Geometry check sheet. Reference: the model listing, model coordinates, mm. A direction names the side the tool comes from. Coordinates: 2 decimals unless noted, no trailing zeros. Write each loop counter-clockwise with the first axis right and the second up, starting at its lowest first coordinate (ties: lowest second). Pieces come first, ordered by that corner, then holes. Notation, with made-up numbers: M -23.75,-3.75 L 0.25,-3.75 A26 cw 0.25,35.25 Z; hole C 5.5,84.5 d4. An arc over 180 degrees is marked long. Put each result on its own line as item: value. Start each with the question number.
1) Scan lines: line 1 along X through (y, z) = (12, 3.25); line 2 along X through (y, z) = (0.25, -5.5); line 3 along Z through (x, y) = (-3, 11.5). Record each from-to range of solid material in increasing order.
2) Gauge pin test, flat ends, axial feed: pin 1 (3 mm diameter, centred on x = 13, z = -3, fed in from +Y); pin 2 (3 mm diameter, centred on x = -18, y = 0, fed in from -Z); pin 3 (6.5 mm diameter, centred on y = 10, z = 0.5, fed in from +X); pin 4 (2.5 mm diameter, centred on y = 10.5, z = 0, fed in from +X). Record the tip position at first contact, or that the pin passes through.
3) Cross-section at C-C on z = -3.5. Record the cut outline in (x, y), plus the area to 3 significant figures.
4) Mould release check, pull along Z, two halves, no side actions. Record for faces 1 (the flat face through (6, 5, 6.5)), 2 (the flat face through (1.9, 12, 2)), 3 (the flat face through (-5, 5, -6.5)): released by +Z, released by -Z, zero draft, split by the parting line, or undercut.
5) Cross-section at D-D on y = 11.5. Record the cut outline in (x, z), plus the area to 3 significant figures.
6) Cross-section at B-B on x = 16.5. Record the cut outline in (y, z), plus the area to 3 significant figures.
7) Cross-section at A-A on y = 0. Record the cut outline in (x, z).
8) Set-up check for faces 4 (the cylindrical face through (1.21, 8.27, 0.29)), 5 (the flat face through (6.5, 15, 0)), 6 (the flat face through (-6.5, 14, 0)), 7 (the flat face through (-0.5, 9.7, 0.1)), 8 (the cylindrical face through (0.45, -12.49, 2.98)): record each of +Z, -Z, +X, -X, +Y, -Y from which the full face is reachable in a straight line by a thin tool's end or side.
from build123d import *
from build123d.topology import SkipClean

# Parameters (mm, degrees)
EXTRUDE_1_DEPTH     = 6.5
EXTRUDE_START       = -7
SKETCH_2_R          = 2.5
EXTRUDE_2_DEPTH     = 7
SKETCH_3_W          = 1.65
SKETCH_3_H          = 23
CUT_EXTRUDE_START   = 10
CUT_EXTRUDE_1_DEPTH = 10


with BuildPart() as part:
    # 草图1 → 凸台-拉伸1 (new, symmetric)
    with BuildSketch(Plane.XY):
        with BuildLine():
            Line((0.5, 5.979130372), (0.5, 15.5))
            Line((0.5, 15.5), (6.5, 15.5))
            Line((6.5, 15.5), (6.5, 10.677078252))
            ThreePointArc((6.5, 10.677078252), (0, -12.5), (-6.5, 10.677078252))
            Line((-6.5, 10.677078252), (-6.5, 15.5))
            Line((-6.5, 15.5), (-0.5, 15.5))
            Line((-0.5, 15.5), (-0.5, 5.979130372))
            ThreePointArc((-0.5, 5.979130372), (0, -6), (0.5, 5.979130372))
        make_face()
    extrude(amount=EXTRUDE_1_DEPTH, both=True)

    # 草图2 → 凸台-拉伸2 (add)
    # profile 1 of 2: a face of its own
    with BuildSketch(Plane(origin=(0, 0, -6.5), x_dir=(-1, 0, 0), z_dir=(0, 0, -1)).offset(EXTRUDE_START)):
        with BuildLine():
            Line((-23.5, -3), (-5.197687408, -11.368115306))
            ThreePointArc((-5.197687408, -11.368115306), (-12.478245567, -0.737148272), (-6.5, 10.677078252))
            Line((-6.5, 10.677078252), (-23.5, 3))
            Line((-23.5, 3), (-23.5, -3))
        make_face()
        with Locations((-18, 0)):
            Circle(SKETCH_2_R, mode=Mode.SUBTRACT)
    # profile 2 of 2: a face of its own
    with BuildSketch(Plane(origin=(0, 0, -6.5), x_dir=(-1, 0, 0), z_dir=(0, 0, -1)).offset(EXTRUDE_START)):
        with BuildLine():
            ThreePointArc((6.5, 10.677078252), (12.478245567, -0.737148272), (5.197687408, -11.368115306))
            Line((5.197687408, -11.368115306), (23.5, -3))
            Line((23.5, -3), (23.5, 3))
            Line((23.5, 3), (6.5, 10.677078252))
        make_face()
        with Locations((18, 0)):
            Circle(SKETCH_2_R, mode=Mode.SUBTRACT)
    extrude(amount=EXTRUDE_2_DEPTH)

    # 草图3 → M4 螺纹孔1 (revolve, cut)
    with BuildSketch(Plane(origin=(-0.5, 11.5, 0), x_dir=(0, 0, -1), z_dir=(0, 1, 0))):
        with Locations((0.825, 11.5)):
            Rectangle(SKETCH_3_W, SKETCH_3_H)
    revolve(axis=Axis((5.85, 11.5, 0), (-1, 0, 0)), mode=Mode.SUBTRACT)

    # 草图5 → 打孔尺寸(%根据)内六角圆柱头螺钉的类型1 (revolve, cut)
    with BuildSketch(Plane(origin=(6.5, 10.5, 0), x_dir=(0, 0, -1), z_dir=(0, 1, 0))):
        Polygon((0, 0), (0, 7.351936393), (2.25, 6), (2.25, 4.6), (4, 4.6), (4, 0), align=None)
    revolve(axis=Axis((12.85, 10.5, 0), (-1, 0, 0)), mode=Mode.SUBTRACT)

    # 草图7 → 切除-拉伸1 (cut)
    with SkipClean():  # the faces are left unmerged after this step: merging them gives an invalid solid
        with BuildSketch(Plane(origin=(6.5, 0, 0), x_dir=(0, 0, -1), z_dir=(1, 0, 0)).offset(CUT_EXTRUDE_START)):
            with BuildLine():
                Line((-0.5, 10.677078252), (-3.996078489, 10.677078252))
                ThreePointArc((-3.996078489, 10.677078252), (0, 6.5), (3.996078489, 10.677078252))
                Line((3.996078489, 10.677078252), (-0.5, 10.677078252))
            make_face()
        extrude(amount=-CUT_EXTRUDE_1_DEPTH, mode=Mode.SUBTRACT)


solid = part.part
Answer key:
1. line 1: x = -6.5 to -0.5, 0.5 to 1.9
1. line 2: x = -23.5 to -20.49, -15.51 to -5.99, 5.99 to 15.51, 20.49 to 23.5
1. line 3: z = -6.5 to -1.65, 1.65 to 6.5
2. pin 1: stops at y = 8.39
2. pin 2: passes through
2. pin 3: stops at x = 1.9
2. pin 4: stops at x = -0.5
3. outline: M -23.5,-3 L -5.2,-11.37 A12.5 ccw 5.2,-11.37 L 23.5,-3 L 23.5,3 L 11.18,8.56 L 1.9,8.56 L 1.9,12.44 L 6.5,12.44 L 6.5,15.5 L 0.5,15.5 L 0.5,5.98 A6 cw long -0.5,5.98 L -0.5,15.5 L -6.5,15.5 L -6.5,10.68 L -23.5,3 Z; hole C -18,0 d5; hole C 18,0 d5
3. area: 638 mm²
4. face 1: released by +Z
4. face 2: undercut
4. face 3: released by -Z
5. outline: M -6.5,-6.5 L -0.5,-6.5 L -0.5,-1.65 L -6.5,-1.65 Z; M -6.5,1.65 L -0.5,1.65 L -0.5,6.5 L -6.5,6.5 Z; M 0.5,-6.5 L 6.5,-6.5 L 6.5,-3.87 L 1.9,-3.87 L 1.9,-2.02 L 0.5,-2.02 Z; M 0.5,2.02 L 1.9,2.02 L 1.9,3.87 L 6.5,3.87 L 6.5,6.5 L 0.5,6.5 Z
5. area: 94.9 mm²
6. outline: M -6.2,-6.5 L -2,-6.5 L -2,0.5 L -6.2,0.5 Z; M 2,-6.5 L 6.16,-6.5 L 6.16,0.5 L 2,0.5 Z
6. area: 58.5 mm²
7. outline: M -23.5,-6.5 L -20.5,-6.5 L -20.5,0.5 L -23.5,0.5 Z; M -15.5,-6.5 L -6,-6.5 L -6,6.5 L -12.5,6.5 L -12.5,0.5 L -15.5,0.5 Z; M 6,-6.5 L 15.5,-6.5 L 15.5,0.5 L 12.5,0.5 L 12.5,6.5 L 6,6.5 Z; M 20.5,-6.5 L 23.5,-6.5 L 23.5,0.5 L 20.5,0.5 Z
8. face 4: +X
8. face 5: +Z, -Z, +X, +Y
8. face 6: +Z, -Z, -X, +Y
8. face 7: +Z, -Z, +Y
8. face 8: +Z
